Geometry: final body of the model. Coordinates: model frame, mm. A direction names the side the tool comes from. Round coordinates to 2 decimals unless told otherwise and drop trailing zeros. Loops run counter-clockwise (first coordinate to the right, second up) from the corner with the lowest first, then second, coordinate; pieces in that order, holes last. Notation, with made-up numbers: (50, 52) - (107, 52) arc R18 cw to (107, 66) - close; hole circle Ø11 at (87.5, 43). An arc over 180 degrees is marked (long way). Answer as CSV lines item,"result".
from build123d import *

# Parameters (mm, degrees)
FLANGE_PROFILE_SKETCH_R   = 6.5
FLANGE_PLATE_20MM_DEPTH   = 20
FLANGE_PROFILE_SKETCH_R_2 = 11.5
FLANGE_PLATE_20MM_2_DEPTH = 20
SQUARE_BOSS_45MM_DEPTH    = 45
BOSS_POCKET_SKETCH_R      = 72.5
BOSS_POCKET_SKETCH_R_2    = 52.5
BOSS_POCKET_CUT_DEPTH     = 3


with BuildPart() as part:
    # Flange Profile Sketch → Flange Plate 20mm (new body)
    with BuildSketch(Plane.XY):
        with BuildLine():
            Line((-89.148145657, 58.529523872), (-78.104184034, 17.312897978))
            ThreePointArc((-78.104184034, 17.312897978), (-80, 0), (-78.104184034, -17.312897978))
            Line((-78.104184034, -17.312897978), (-89.148145657, -58.529523872))
            ThreePointArc((-89.148145657, -58.529523872), (-82.677671147, -82.677667913), (-58.52952829, -89.148146841))
            Line((-58.52952829, -89.148146841), (-17.312897978, -78.104184034))
            ThreePointArc((-17.312897978, -78.104184034), (-8.453e-06, -80), (17.312881472, -78.104187693))
            Line((17.312881472, -78.104187693), (58.52952829, -89.148146841))
            ThreePointArc((58.52952829, -89.148146841), (82.677672617, -82.677669383), (89.148145657, -58.529523872))
            Line((89.148145657, -58.529523872), (78.104184034, -17.312897978))
            ThreePointArc((78.104184034, -17.312897978), (80, 0), (78.104184034, 17.312897978))
            Line((78.104184034, 17.312897978), (89.148145657, 58.529523872))
            ThreePointArc((89.148145657, 58.529523872), (82.67767031, 82.677667076), (58.52952829, 89.148146841))
            Line((58.52952829, 89.148146841), (17.312897978, 78.104184034))
            ThreePointArc((17.312897978, 78.104184034), (8.453e-06, 80), (-17.312881472, 78.104187693))
            Line((-17.312881472, 78.104187693), (-58.52952829, 89.148146841))
            ThreePointArc((-58.52952829, 89.148146841), (-82.677671147, 82.677667913), (-89.148145657, 58.529523872))
        make_face()
        with Locations((-65, -65)):
            Circle(FLANGE_PROFILE_SKETCH_R, mode=Mode.SUBTRACT)
        with Locations((65.00000294, -65.00000294)):
            Circle(FLANGE_PROFILE_SKETCH_R, mode=Mode.SUBTRACT)
        with Locations((64.999998327, 64.999998327)):
            Circle(FLANGE_PROFILE_SKETCH_R, mode=Mode.SUBTRACT)
        with Locations((-65, 65)):
            Circle(FLANGE_PROFILE_SKETCH_R, mode=Mode.SUBTRACT)
        with BuildLine():
            Line((-50, -35), (-50, 35))
            ThreePointArc((-50, 35), (-45.606601718, 45.606601718), (-35, 50))
            Line((-35, 50), (35, 50))
            ThreePointArc((35, 50), (45.606601718, 45.606601718), (50, 35))
            Line((50, 35), (50, -35))
            ThreePointArc((50, -35), (45.606601718, -45.606601718), (35, -50))
            Line((35, -50), (-35, -50))
            ThreePointArc((-35, -50), (-45.606601718, -45.606601718), (-50, -35))
        make_face(mode=Mode.SUBTRACT)
    extrude(amount=FLANGE_PLATE_20MM_DEPTH)



with BuildPart() as body_2:
    # Flange Profile Sketch → Flange Plate 20mm 2 (new body)
    with BuildSketch(Plane.XY):
        with BuildLine():
            ThreePointArc((-44, 29), (-39.606601718, 39.606601718), (-29, 44))
            Line((-29, 44), (29, 44))
            ThreePointArc((29, 44), (39.606601718, 39.606601718), (44, 29))
            Line((44, 29), (44, -29))
            ThreePointArc((44, -29), (39.606601718, -39.606601718), (29, -44))
            Line((29, -44), (-29, -44))
            ThreePointArc((-29, -44), (-39.606601718, -39.606601718), (-44, -29))
            Line((-44, -29), (-44, 29))
        make_face()
        with Locations((-22, 22)):
            Circle(FLANGE_PROFILE_SKETCH_R_2, mode=Mode.SUBTRACT)
        with Locations((22, 22)):
            Circle(FLANGE_PROFILE_SKETCH_R_2, mode=Mode.SUBTRACT)
        with Locations((22, -22)):
            Circle(FLANGE_PROFILE_SKETCH_R_2, mode=Mode.SUBTRACT)
        with Locations((-22, -22)):
            Circle(FLANGE_PROFILE_SKETCH_R_2, mode=Mode.SUBTRACT)
    extrude(amount=FLANGE_PLATE_20MM_2_DEPTH)


with BuildPart() as part_1:
    add(part.part)

    add(body_2.part)  # Square Boss 45mm merges body 2
    # Sketch2_6 → Square Boss 45mm (add)
    with BuildSketch(Plane.XY):
        with BuildLine():
            ThreePointArc((-50, 35), (-45.606601718, 45.606601718), (-35, 50))
            Line((-35, 50), (35, 50))
            ThreePointArc((35, 50), (45.606601718, 45.606601718), (50, 35))
            Line((50, 35), (50, -35))
            ThreePointArc((50, -35), (45.606601718, -45.606601718), (35, -50))
            Line((35, -50), (-35, -50))
            ThreePointArc((-35, -50), (-45.606601718, -45.606601718), (-50, -35))
            Line((-50, -35), (-50, 35))
        make_face()
        with BuildLine():
            Line((-44, -29), (-44, 29))
            ThreePointArc((-44, 29), (-39.606601718, 39.606601718), (-29, 44))
            Line((-29, 44), (29, 44))
            ThreePointArc((29, 44), (39.606601718, 39.606601718), (44, 29))
            Line((44, 29), (44, -29))
            ThreePointArc((44, -29), (39.606601718, -39.606601718), (29, -44))
            Line((29, -44), (-29, -44))
            ThreePointArc((-29, -44), (-39.606601718, -39.606601718), (-44, -29))
        make_face(mode=Mode.SUBTRACT)
    extrude(amount=SQUARE_BOSS_45MM_DEPTH)

    # Boss Pocket Sketch → Boss Pocket Cut (cut)
    with BuildSketch(Plane(origin=(0, 0, 0), x_dir=(-1, 0, 0), z_dir=(0, 0, -1))):
        Circle(BOSS_POCKET_SKETCH_R)
        Circle(BOSS_POCKET_SKETCH_R_2, mode=Mode.SUBTRACT)
    extrude(amount=-BOSS_POCKET_CUT_DEPTH, mode=Mode.SUBTRACT)


solid = part_1.part
(1) Pin query (flat end, axial travel): P1, Ø7.5, axis at x = 3, z = 37, coming from the +Y side; P2, Ø1.5, axis at y = -5.5, z = 10.5, coming from the +X side; P3, Ø20, axis at y = 1, z = 31, coming from the +X side. Return the tip coordinate at first contact, or that it passes through.
Findings below:
P1,"y = 50"
P2,"x = 79.86"
P3,"x = 50"
(2) Section A-A (z = 11.5). Give the number of separate pieces and of enclosed holes in the cut face, and give its area (3 significant figures).
Findings below:
separate pieces,"1"
enclosed holes,"8"
area,"26,100 mm2"
(3) Draft query along X for faces 1 (the face through (-62.001, -70.767, 9.86)), 2 (the face through (73, -6, 0)), 3 (the face through (83.55, 37.63, 9.86)). Return one class per face: pulls with the +X half, pulls with the -X half, needs draft (parallel to the pull), parting line crosses it, or undercut.
Findings below:
face 1,"undercut"
face 2,"needs draft"
face 3,"pulls with the +X half"
(4) Access query for faces 4 (the face through (83.7, -38.2, 9.9)), 5 (the face through (39.49, 39.72, 32.33)), 6 (the face through (-83.7, 38.2, 9.9)), 7 (the face through (-38.2, -83.7, 9.9)). Directions: +Z, -Z, +X, -X, +Y, -Y. A direction counts if a zero-diameter tool reaches every point of the face in a straight line with its end or side. Return the directions, or none.
Findings below:
face 4,"+Z, -Z, +X"
face 5,"+Z"
face 6,"+Z, -Z, -X"
face 7,"+Z, -Z, -Y"
(5) Section B-B (y = 26). Output: boundary loops of the cut face in (x, z).
Findings below:
outline,"(-80.43, 0) - (-67.68, 0) - (-67.68, 3) - (-45.61, 3) - (-45.61, 0) - (-32.78, 0) - (-32.78, 20) - (-44, 20) - (-44, 45) - (-50, 45) - (-50, 20) - (-80.43, 20) - close; (-11.22, 0) - (11.22, 0) - (11.22, 20) - (-11.22, 20) - close; (32.78, 0) - (45.61, 0) - (45.61, 3) - (67.68, 3) - (67.68, 0) - (80.43, 0) - (80.43, 20) - (50, 20) - (50, 45) - (44, 45) - (44, 20) - (32.78, 20) - close"
(6) Material intervals for line 1 along Y through (x, z) = (-65, 11.75); line 2 along Y through (x, z) = (0, 1.9); line 3 along X through (y, z) = (-6.5, 23.5), sorted ascending.
Findings below:
line 1,"-90 to -71.5, -58.5 to 58.5, 71.5 to 90"
line 2,"-80 to -72.5, -52.5 to 52.5, 72.5 to 80"
line 3,"-50 to -44, 44 to 50"
(7) Section D-D (x = 22). Output: boundary loops of the cut face in (y, z), and give its area (3 significant figures).
Findings below:
outline,"(-79.36, 0) - (-69.08, 0) - (-69.08, 3) - (-47.67, 3) - (-47.67, 0) - (-33.5, 0) - (-33.5, 20) - (-44, 20) - (-44, 45) - (-50, 45) - (-50, 20) - (-79.36, 20) - close; (-10.5, 0) - (10.5, 0) - (10.5, 20) - (-10.5, 20) - close; (33.5, 0) - (47.67, 0) - (47.67, 3) - (69.08, 3) - (69.08, 0) - (79.36, 0) - (79.36, 20) - (50, 20) - (50, 45) - (44, 45) - (44, 20) - (33.5, 20) - close"
area,"2,430 mm2"
(8) Section C-C (z = 25). Output: boundary loops of the cut face in (x, y), and give its area (3 significant figures).
Findings below:
outline,"(-50, -35) arc R15 ccw to (-35, -50) - (35, -50) arc R15 ccw to (50, -35) - (50, 35) arc R15 ccw to (35, 50) - (-35, 50) arc R15 ccw to (-50, 35) - close; hole (-44, -29) arc R15 ccw to (-29, -44) - (29, -44) arc R15 ccw to (44, -29) - (44, 29) arc R15 ccw to (29, 44) - (-29, 44) arc R15 ccw to (-44, 29) - close"
area,"2,260 mm2"
